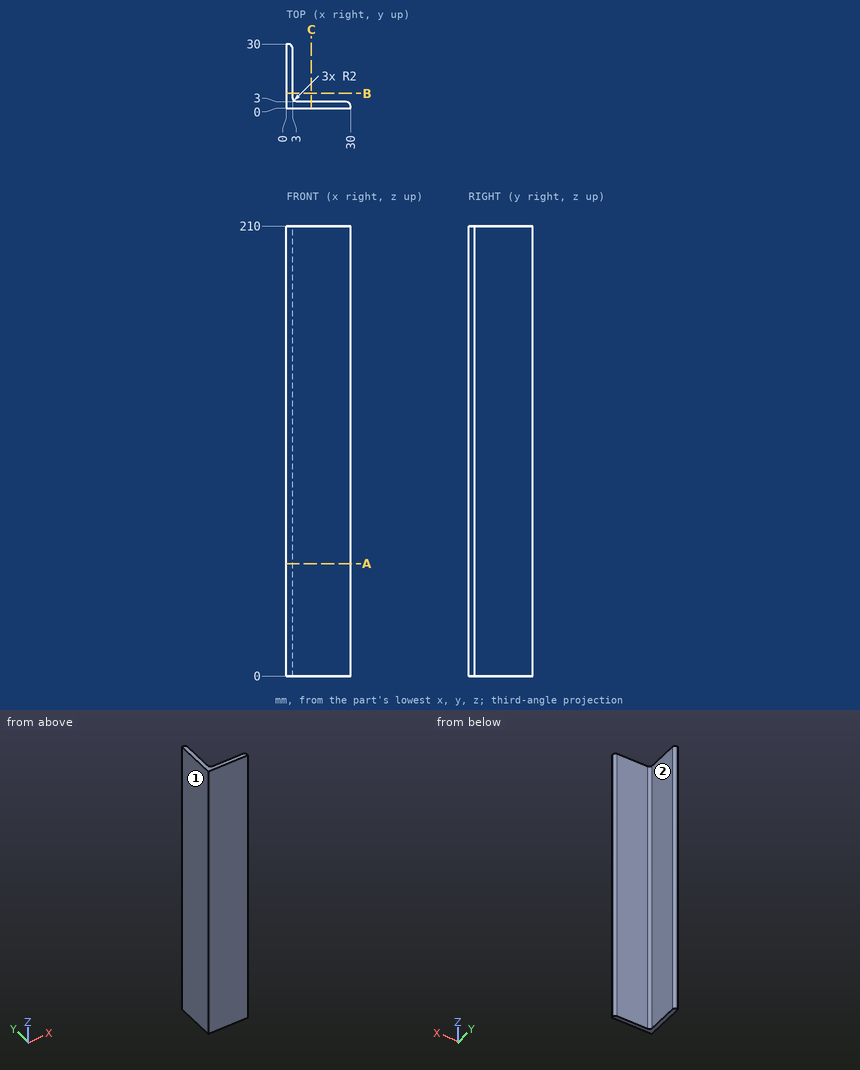
Can you work these out from the drawing? Everything is in mm from the part's minimum corner. A direction names the side the tool comes from. Round coordinates to 2 decimals unless told otherwise and drop trailing zeros. Write each loop counter-clockwise with the first axis right and the second up, starting at its lowest first coordinate (ties: lowest second). Pieces come first, ordered by that corner, then holes. Notation, with made-up numbers: (-15, 89.25) - (17, 89.25) arc R34 ccw to (17, 125.25) - close; hole circle Ø5 at (57, -10). An arc over 180 degrees is marked (long way). Use a Markdown table: item, result.
Q1. I want a section at A-A (z = 52.5). List the corners of the cut face in (x, y) for me, plus the area to 3 significant figures.
Output values:
| item | result |
|---|---|
| outline | (0, 0) - (30, 0) - (30, 1) arc R2 ccw to (28, 3) - (5, 3) arc R2 cw to (3, 5) - (3, 28) arc R2 ccw to (1, 30) - (0, 30) - close |
| area | 170 mm2 |
Q2. I want a section at B-B (y = 7). List the corners of the cut face in (x, z) for me, plus the area to 3 significant figures.
Output values:
| item | result |
|---|---|
| outline | (0, 0) - (3, 0) - (3, 210) - (0, 210) - close |
| area | 630 mm2 |
Q3. Please list where these lines run through material, in increasing order: L1, parallel to X at y = 24.25, z = 108.5; L2, parallel to Y at x = 2, z = 147.
Output values:
| item | result |
|---|---|
| L1 | 0 to 3 |
| L2 | 0 to 29.73 |
Q4. For the marked faces 1 and 2, which set-ups out of +Z, -Z, +X, -X, +Y, -Y let a thin tool reach every point of the face, with its end or its side?
Output values:
| item | result |
|---|---|
| face 1 | +Z, -Z, -X, +Y, -Y |
| face 2 | +Z, -Z, +X, +Y |
Q5. For pin 1 (5 mm diameter, centred on x = 7, y = 27, fed in from -Z); pin 2 (7 mm diameter, centred on x = 20.5, z = 94, fed in from +Y), each with a flat end and sliding along its axis, tell me the tip position at first contact or that it passes through.
Output values:
| item | result |
|---|---|
| pin 1 | through |
| pin 2 | y = 3 |
